Work out the finished part from the listing and answer in its coordinate system (mm). A direction names the side the tool comes from. Round coordinates to 2 decimals unless told otherwise and drop trailing zeros. Loops run counter-clockwise (first coordinate to the right, second up) from the corner with the lowest first, then second, coordinate; pieces in that order, holes last.
```python
from build123d import *

# Parameters (mm, degrees)
SKETCH_1_W                   = 15
SKETCH_1_H                   = 15.8
EXTRUDE_1_DEPTH              = 4.5
HOLE_WIZARD_M4_1_D           = 5.5
HOLE_WIZARD_M4_1_CBORE_D     = 10
HOLE_WIZARD_M4_1_CBORE_DEPTH = 5.7
CUT_EXTRUDE_1_DEPTH          = 18.540239451


with BuildPart() as part:
    # 草图1 → 凸台-拉伸1 (new, symmetric)
    with BuildSketch(Plane.XY):
        Rectangle(SKETCH_1_W, SKETCH_1_H)
    extrude(amount=EXTRUDE_1_DEPTH, both=True)

    # M4 沉头孔1 (through all)
    with Locations(Plane.XY.offset(4.5)):
        with Locations((0, 0)):
            CounterBoreHole(HOLE_WIZARD_M4_1_D / 2, HOLE_WIZARD_M4_1_CBORE_D / 2, HOLE_WIZARD_M4_1_CBORE_DEPTH)

    # 草图4 → 切除-拉伸1 (cut, through all)
    with BuildSketch(Plane(origin=(7.5, 0, 0), x_dir=(0, 0, -1), z_dir=(1, 0, 0))):
        Polygon((-4.5, -7.9), (-4.5, -5.4), (-1.5, -7.9), align=None)
        Polygon((-4.5, 5.4), (-4.5, 7.9), (-1.5, 7.9), align=None)
    extrude(amount=-CUT_EXTRUDE_1_DEPTH, mode=Mode.SUBTRACT)


solid = part.part
```
1. Find section A-A (y = 0). Write down the section's boundary in (x, z), then the cut area to 4 significant figures.
Answer key:
outline: (-7.5, -4.5) - (-2.75, -4.5) - (-2.75, -1.2) - (-5, -1.2) - (-5, 4.5) - (-7.5, 4.5) - close; (2.75, -4.5) - (7.5, -4.5) - (7.5, 4.5) - (5, 4.5) - (5, -1.2) - (2.75, -1.2) - close
area: 59.85 mm2
2. Which of the six approach directions +Z, -Z, +X, -X, +Y, -Y give full straight-line access (tool end or side, diameter ignored) to faces 5 (the face through (-3, 0, -4.5)), 6 (the face through (2.2, -2.2, -1.2))?
Answer key:
face 5: -Z, +X, -X, +Y, -Y
face 6: +Z
3. Find section C-C (z = -2.25). Write down the section's boundary in (x, y), then the cut area to 3 significant figures.
Answer key:
outline: (-7.5, -7.9) - (7.5, -7.9) - (7.5, 7.9) - (-7.5, 7.9) - close; hole circle Ø5.5 at (0, 0)
area: 213 mm2
4. Find section B-B (x = 0). Write down the section's boundary in (y, z).
Answer key:
outline: (-7.9, -4.5) - (-2.75, -4.5) - (-2.75, -1.2) - (-5, -1.2) - (-5, 4.5) - (-5.4, 4.5) - (-7.9, 1.5) - close; (2.75, -4.5) - (7.9, -4.5) - (7.9, 1.5) - (5.4, 4.5) - (5, 4.5) - (5, -1.2) - (2.75, -1.2) - close
5. Find section D-D (x = -4.25). Write down the section's boundary in (y, z), then the cut area to 3 significant figures.
Answer key:
outline: (-7.9, -4.5) - (7.9, -4.5) - (7.9, 1.5) - (5.4, 4.5) - (2.63, 4.5) - (2.63, -1.2) - (-2.63, -1.2) - (-2.63, 4.5) - (-5.4, 4.5) - (-7.9, 1.5) - close
area: 105 mm2
6. Consider probe 1 along Y at (x, z) = (0, -2.75); probe 2 along Y at (x, z) = (0, 1); probe 3 along X at (y, z) = (3.5, 4.25). Determine where each line is inside the solid, lowest interval first.
Answer key:
probe 1: y = -7.9 to -2.75, 2.75 to 7.9
probe 2: y = -7.9 to -5, 5 to 7.9
probe 3: x = -7.5 to -3.57, 3.57 to 7.5
7. Determine the mould class of faces 1 (the face through (7.5, 0, 0)), 2 (the face through (0, 7.9, -1)), 3 (the face through (0.596, -2.685, -2.873)), 4 (the face through (-1.08, -4.88, 1.69)) for opening direction X: +X half, -X half, draft (parallel to the pull), parting line (faces both ways), or undercut.
Answer key:
face 1: +X half
face 2: draft
face 3: undercut
face 4: undercut
